For this review, take the finished solid that the model builds, in its own axes (mm). Coordinates: 2 decimals unless noted, no trailing zeros. Loops run counter-clockwise (first coordinate to the right, second up) from the corner with the lowest first, then second, coordinate; pieces in that order, holes last. Notation, with made-up numbers: M -15,65.5 L 41,65.5 A28 cw 41,89.5 Z; hole C 22,88 d1. An arc over 180 degrees is marked long. Put each result on its own line as item: value.
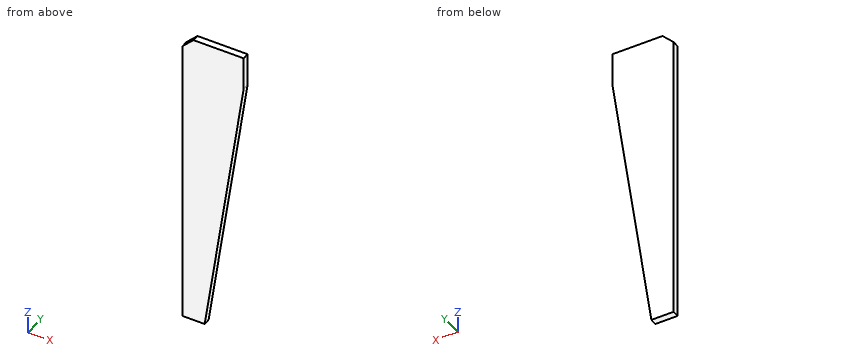
```python
from build123d import *

# Parameters (mm, degrees)
BOSS_EXTRUDE1_DEPTH = 6
CHAMFER1_SIZE       = 20


with BuildPart() as part:
    # Sketch1 → Boss-Extrude1 (new, symmetric)
    with BuildSketch(Plane(origin=(0, 0, 0), x_dir=(1, 0, 0), z_dir=(0, 1, 0))):
        Polygon((-20, 20), (-20, 550), (20, 550), (90, 60), (90, 0), (0, 0), (-20, 0), align=None)
    extrude(amount=BOSS_EXTRUDE1_DEPTH, both=True)

    # Chamfer1
    chamfer1_edges = [part.edges().sort_by_distance(p)[0] for p in [
        (-20, 0, 0),
    ]]
    chamfer(chamfer1_edges, length=CHAMFER1_SIZE)


solid = part.part
```
(1) Add section C-C (z = -189.5). Write out the cut boundary in (x, y), plus the area to 3 significant figures.
Determined:
outline: M -20,-6 L 71.5,-6 L 71.5,6 L -20,6 Z
area: 1,100 mm^2
(2) For pin 1 (3 mm diameter, centred on y = -1.5, z = -236, fed in from +X), flat-tipped, find the tip position at first contact; note if it passes through.
Determined:
pin 1: stops at x = 65.07
(3) Add section B-B (x = -9). Write out the cut boundary in (y, z), plus the area to 3 significant figures.
Determined:
outline: M -6,-550 L 6,-550 L 6,-9 L -6,-9 Z
area: 6,490 mm^2
(4) Add section A-A (y = -1.75). Write out the cut boundary in (x, z), plus the area to 4 significant figures.
Determined:
outline: M -20,-550 L 20,-550 L 90,-60 L 90,0 L 0,0 L -20,-20 Z
area: 43,150 mm^2
(5) Wall thickness on line 1 along X through (y, z) = (-0.75, -215.5); line 2 along X through (y, z) = (-3.25, -430); line 3 along Z through (x, y) = (-5.5, -3.5): over which ranges is each line inside the solid? List them lowest first. Write a range as [from, to].
Determined:
line 1: x = [-20, 67.79]
line 2: x = [-20, 37.14]
line 3: z = [-550, -5.5]
